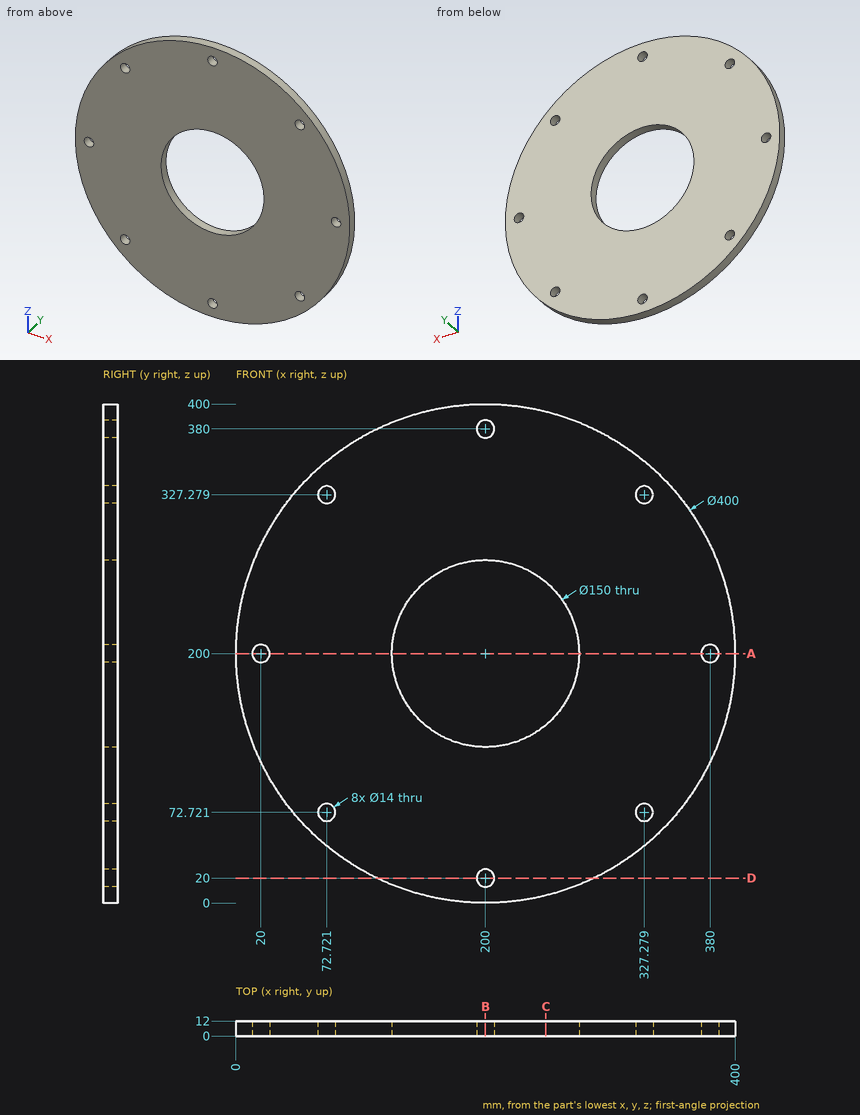
Geometry check sheet. Reference: drawing and pictorial views, mm from the part's lowest x, y, z. Give positions to 0.01 mm unless a question says otherwise; leave off trailing zeros. Write each loop counter-clockwise with the first axis right and the second up, starting at its lowest first coordinate (ties: lowest second). Pieces come first, ordered by that corner, then holes.
Item 1: Cross-section at D-D (z = 20). Enter the section's corners in (x, y).
Item 2: Cross-section at A-A (z = 200). Enter the section's corners in (x, y), and give its area (3 significant figures).
Item 3: Scan lines: L1, parallel to X at y = 3.5, z = 200; L2, parallel to Z at x = 322, y = 1.25 (1 decimal); L3, parallel to X at y = 9.25, z = 196 (1 decimal). Record each from-to range of solid material in increasing order.
Item 4: Cross-section at B-B (x = 200). Enter the section's corners in (y, z), and give its area (3 significant figures).
Item 5: Cross-section at C-C (x = 248.5). Enter the section's corners in (y, z).
Item 6: Gauge pin test, flat ends, axial feed: pin 1 (4 mm diameter, centred on x = 49, y = 6, fed in from -Z); pin 2 (12 mm diameter, centred on x = 244, z = 87.5, fed in from -Y); pin 3 (6 mm diameter, centred on y = 1.5, z = 278, fed in from -X) (1 decimal); pin 4 (6 mm diameter, centred on x = 122, y = 3.5, fed in from +Z) (1 decimal). Record the tip position at first contact, or that the pin passes through.
Report:
1. outline: (112.82, 0) - (193, 0) - (193, 12) - (112.82, 12) - close; (207, 0) - (287.18, 0) - (287.18, 12) - (207, 12) - close
2. outline: (0, 0) - (13, 0) - (13, 12) - (0, 12) - close; (27, 0) - (125, 0) - (125, 12) - (27, 12) - close; (275, 0) - (373, 0) - (373, 12) - (275, 12) - close; (387, 0) - (400, 0) - (400, 12) - (387, 12) - close
2. area: 2,660 mm2
3. L1: x = 0 to 13, 27 to 125, 275 to 373, 387 to 400
3. L2: z = 41.5 to 68.1, 77.3 to 322.7, 331.9 to 358.5
3. L3: x = 0 to 14.3, 25.7 to 125.1, 274.9 to 374.3, 385.7 to 400
4. outline: (0, 0) - (12, 0) - (12, 13) - (0, 13) - close; (0, 27) - (12, 27) - (12, 125) - (0, 125) - close; (0, 275) - (12, 275) - (12, 373) - (0, 373) - close; (0, 387) - (12, 387) - (12, 400) - (0, 400) - close
4. area: 2,660 mm2
5. outline: (0, 5.97) - (12, 5.97) - (12, 142.79) - (0, 142.79) - close; (0, 257.21) - (12, 257.21) - (12, 394.03) - (0, 394.03) - close
6. pin 1: stops at z = 66.59
6. pin 2: stops at y = 0
6. pin 3: stops at x = 14.6
6. pin 4: stops at z = 385.4
